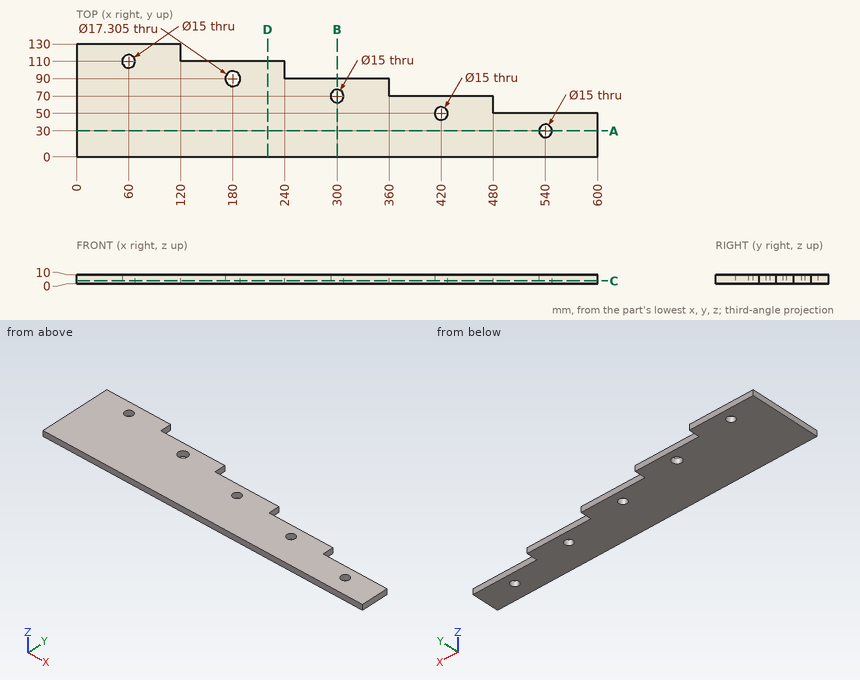
Part print with two shaded views. Sizes in mm from the minimum x, y, z corner. Round coordinates to 2 decimals unless told otherwise and drop trailing zeros. Loops run counter-clockwise (first coordinate to the right, second up) from the corner with the lowest first, then second, coordinate; pieces in that order, holes last. Notation, with made-up numbers: M -29,-39.75 L 21,-39.75 A25 ccw 21,-1.75 Z; hole C 26.5,43 d10. An arc over 180 degrees is marked long. Return JSON: item names as keys, results as strings. Group by question number.
(1) Saw through at A-A, the plane y = 30. List the corners of the cut face in (x, z), and give its area (3 significant figures).
(2) Saw through at C-C, the plane z = 3. List the corners of the cut face in (x, y) (1 decimal).
(3) Drop flat-ended pins along their axis: P1, Ø3, axis at x = 543.5, z = 6, coming from the +Y side; P2, Ø5, axis at y = 82, z = 3, coming from the +X side; P3, Ø3, axis at x = 301.5, z = 6.5, coming from the +Y side. Give the stop position or say it passes through.
(4) Saw through at D-D, the plane x = 220. List the corners of the cut face in (y, z).
(5) Wall check: probe 1 along X at (y, z) = (50.5, 4.25); probe 2 along Y at (x, z) = (420, 7); probe 3 along Y at (x, z) = (180, 8.25). Give the ranges that are in metal, low to high. Write a range as [from, to].
(6) Saw through at B-B, the plane x = 300. List the corners of the cut face in (y, z).
Answer list:
{
 "1": {"outline": "M 0,0 L 532.5,0 L 532.5,10 L 0,10 Z; M 547.5,0 L 600,0 L 600,10 L 547.5,10 Z", "area": "5,850 mm2"},
 "2": {"outline": "M 0,0 L 600,0 L 600,50 L 480,50 L 480,70 L 360,70 L 360,90 L 240,90 L 240,110 L 120,110 L 120,130 L 0,130 Z; hole C 60,110 d15; hole C 180,90 d17.3; hole C 300,70 d15; hole C 420,50 d15; hole C 540,30 d15"},
 "3": {"P1": "y = 50", "P2": "x = 360", "P3": "y = 90"},
 "4": {"outline": "M 0,0 L 110,0 L 110,10 L 0,10 Z"},
 "5": {"probe 1": "[0, 412.52], [427.48, 480]", "probe 2": "[0, 42.5], [57.5, 70]", "probe 3": "[0, 81.35], [98.65, 110]"},
 "6": {"outline": "M 0,0 L 62.5,0 L 62.5,10 L 0,10 Z; M 77.5,0 L 90,0 L 90,10 L 77.5,10 Z"}
}
